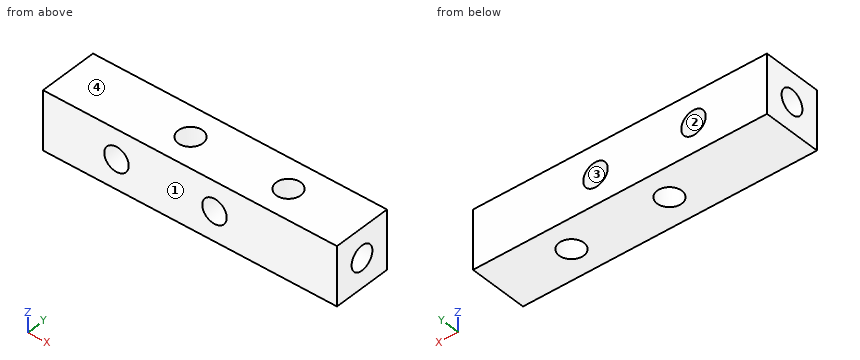
```python
from build123d import *

# Parameters (mm, degrees)
SKETCH_1_W             = 30
SKETCH_1_H             = 6
EXTRUDE_1_DEPTH        = 6
HOLE_WIZARD_M3_1_D     = 2.5
HOLE_WIZARD_M3_2_D     = 2.5
HOLE_WIZARD_M3_3_D     = 2.5
HOLE_WIZARD_M3_3_DEPTH = 4.248924226
HOLE_WIZARD_M3_3_TIP   = 0.751075774
HOLE_WIZARD_M3_4_D     = 2.5
HOLE_WIZARD_M3_4_DEPTH = 4.248924226
HOLE_WIZARD_M3_4_TIP   = 0.751075774


with BuildPart() as part:
    # 草图1 → 凸台-拉伸1 (new body)
    with BuildSketch(Plane(origin=(0, 0, 0), x_dir=(1, 0, 0), z_dir=(0, 1, 0))):
        Rectangle(SKETCH_1_W, SKETCH_1_H)
    extrude(amount=EXTRUDE_1_DEPTH)

    # M3 螺纹孔1 (through all)
    with Locations(Plane.XY.offset(3)):
        with Locations((-2.5, 3), (7.5, 3)):
            Hole(HOLE_WIZARD_M3_1_D / 2)

    # M3 螺纹孔2 (through all)
    with Locations(Plane(origin=(0, 6, 0), x_dir=(1, 0, 0), z_dir=(0, 1, 0))):
        with Locations((2.5, 0), (-7.5, 0)):
            Hole(HOLE_WIZARD_M3_2_D / 2)

    # M3 螺纹孔3
    with Locations(Plane.ZY.offset(15)):
        with Locations((0, 3)):
            Hole(HOLE_WIZARD_M3_3_D / 2, depth=HOLE_WIZARD_M3_3_DEPTH)
            with Locations((0, 0, -(HOLE_WIZARD_M3_3_DEPTH + HOLE_WIZARD_M3_3_TIP / 2))):  # 118° drill point
                Cone(0, HOLE_WIZARD_M3_3_D / 2, HOLE_WIZARD_M3_3_TIP, mode=Mode.SUBTRACT)

    # M3 螺纹孔4
    with Locations(Plane(origin=(15, 0, 0), x_dir=(0, 0, -1), z_dir=(1, 0, 0))):
        with Locations((0, 3)):
            Hole(HOLE_WIZARD_M3_4_D / 2, depth=HOLE_WIZARD_M3_4_DEPTH)
            with Locations((0, 0, -(HOLE_WIZARD_M3_4_DEPTH + HOLE_WIZARD_M3_4_TIP / 2))):  # 118° drill point
                Cone(0, HOLE_WIZARD_M3_4_D / 2, HOLE_WIZARD_M3_4_TIP, mode=Mode.SUBTRACT)


solid = part.part
```
The listing builds one solid part. Answer for the finished solid, in the listing's coordinates (mm). Face numbers are marked on the shaded views. Give positions to 0.01 mm unless a question says otherwise; leave off trailing zeros. Order: outer loops, then holes, each group sorted by start corner. A loop starts at its lowest first (then second) coordinate and runs counter-clockwise, first axis right, second up.
1) Consider line 1 along X through (y, z) = (3.8, 0.7); line 2 along Z through (x, y) = (-7.5, 3.7); line 3 along Y through (x, z) = (12.25, 0). Determine where each line is inside the solid, lowest interval first.
Reported:
line 1: x = -10.64 to -8.54, -6.46 to -3.46, -1.54 to 1.46, 3.54 to 6.54, 8.46 to 10.64
line 2: z = -3 to -1.25, 1.25 to 3
line 3: y = 0 to 1.75, 4.25 to 6
2) Find section C-C on y = 1.5. Write down the section's boundary in (x, z), then the cut area to 3 significant figures.
Reported:
outline: (-15, -3) - (15, -3) - (15, 3) - (-15, 3) - close; hole circle Ø2.5 at (-7.5, 0); hole circle Ø2.5 at (2.5, 0)
area: 170 mm2
3) Find section D-D on x = 11.25. Write down the section's boundary in (y, z).
Reported:
outline: (0, -3) - (6, -3) - (6, 3) - (0, 3) - close; hole circle Ø2.5 at (3, 0)
4) Find section A-A on x = 2.5. Write down the section's boundary in (y, z).
Reported:
outline: (0, -3) - (6, -3) - (6, -1.25) - (0, -1.25) - close; (0, 1.25) - (6, 1.25) - (6, 3) - (0, 3) - close
5) Determine the mould class of the marked faces 1, 2, 3 and 4 for opening direction Z: pulls with the +Z half, pulls with the -Z half, needs draft (parallel to the pull), parting line crosses it, or undercut.
Reported:
face 1: needs draft
face 2: undercut
face 3: undercut
face 4: pulls with the +Z half
6) Find section B-B on z = 1.8. Write down the section's boundary in (x, y), then the cut area to 3 significant figures.
Reported:
outline: (-15, 0) - (15, 0) - (15, 6) - (-15, 6) - close; hole circle Ø2.5 at (-2.5, 3); hole circle Ø2.5 at (7.5, 3)
area: 170 mm2
7) Given P1, Ø2, axis at y = 3, z = 0, coming from the -X side, flat-ended and moving along its own axis, determine where the tip first touches the part or whether it passes through.
Reported:
P1: stops at x = -10.6
